Design review of the part shown in the three views and the two pictorial views. Dimensions are in mm from the part's minimum x, y and z. Round coordinates to 2 decimals unless told otherwise and drop trailing zeros. Order: outer loops, then holes, each group sorted by start corner. A loop starts at its lowest first (then second) coordinate and runs counter-clockwise, first axis right, second up.
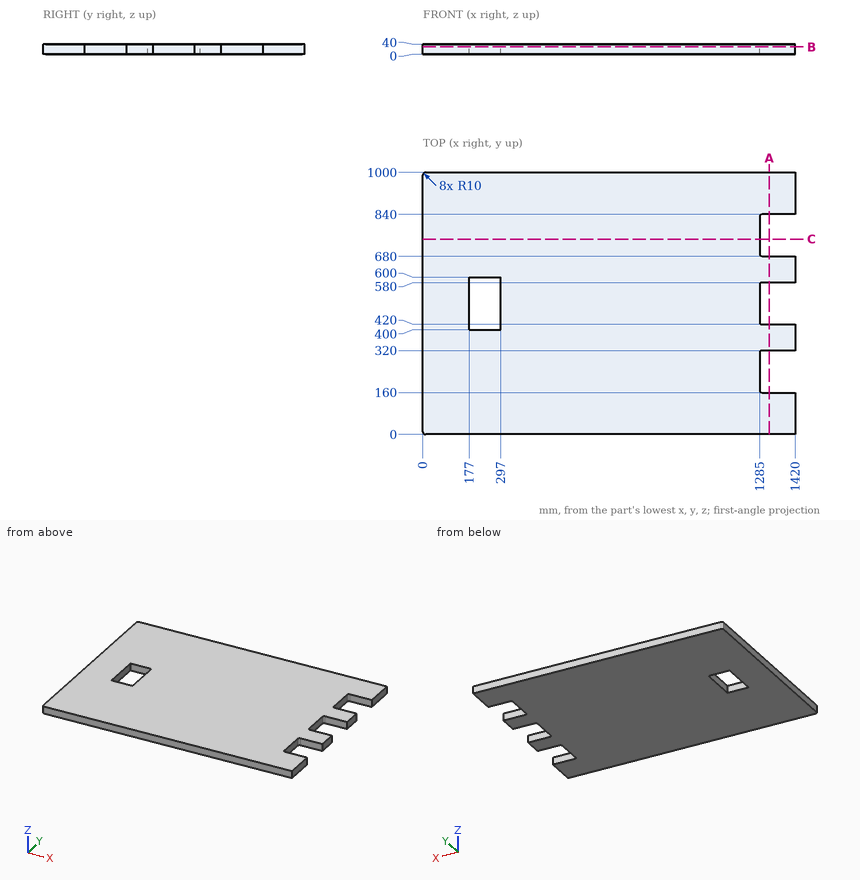
(1) Add section A-A on x = 1322.5. Give the boundary of the cut face in (y, z).
(2) Add section B-B on z = 29. Give the boundary of the cut face in (x, y), plus the area to 3 significant figures.
(3) Add section C-C on y = 745.5. Give the boundary of the cut face in (x, z), plus the area to 3 significant figures.
(4) Wall thickness on L1, parallel to Y at x = 266, z = 27; L2, parallel to X at y = 470, z = 26.5; L3, parallel to X at y = 798, z = 19.5: over which ranges is each line inside the solid? List them lowest first.
(5) Clearance check with flat-ended pins moving along their axes: P1, Ø10, axis at y = 664, z = 21.5, coming from the -X side; P2, Ø12, axis at y = 488.5, z = 12.5, coming from the +X side. State where each tip first meets the part, or that it passes through.
Here are the results:
1. outline: (0, 0) - (160, 0) - (160, 40) - (0, 40) - close; (320, 0) - (420, 0) - (420, 40) - (320, 40) - close; (580, 0) - (680, 0) - (680, 40) - (580, 40) - close; (840, 0) - (1000, 0) - (1000, 40) - (840, 40) - close
2. outline: (0, 10) arc R10 ccw to (10, 0) - (1420, 0) - (1420, 160) - (1295, 160) arc R10 cw to (1285, 170) - (1285, 310) arc R10 cw to (1295, 320) - (1420, 320) - (1420, 420) - (1295, 420) arc R10 cw to (1285, 430) - (1285, 570) arc R10 cw to (1295, 580) - (1420, 580) - (1420, 680) - (1295, 680) arc R10 cw to (1285, 690) - (1285, 830) arc R10 cw to (1295, 840) - (1420, 840) - (1420, 1000) - (10, 1000) arc R10 ccw to (0, 990) - close; hole (177, 400) - (297, 400) - (297, 600) - (177, 600) - close
2. area: 1,330,000 mm2
3. outline: (0, 0) - (1285, 0) - (1285, 40) - (0, 40) - close
3. area: 51,400 mm2
4. L1: y = 0 to 400, 600 to 1000
4. L2: x = 0 to 177, 297 to 1285
4. L3: x = 0 to 1285
5. P1: stops at x = 0
5. P2: stops at x = 1285
